from build123d import *

# Parameters (mm, degrees)
CUT_EXTRUDE1_DEPTH = 261.839989265
CHAMFER1_SIZE      = 2
FILLET1_R          = 0.5


with BuildPart() as part:
    # Sketch1 → Revolve1 (revolve)
    with BuildSketch(Plane.XY, mode=Mode.PRIVATE) as revolve1_sk:
        with BuildLine():
            Line((-125, 122.5), (-116.767790327, 122.5))
            Line((-116.767790327, 122.5), (-10.2606043, 83.734554551))
            ThreePointArc((-10.2606043, 83.734554551), (0, 81.925333174), (10.2606043, 83.734554551))
            Line((10.2606043, 83.734554551), (116.767790327, 122.5))
            Line((116.767790327, 122.5), (125, 122.5))
            Line((125, 122.5), (125, 88.250057247))
            Line((125, 88.250057247), (64.082356705, 66.077848346))
            ThreePointArc((64.082356705, 66.077848346), (59.582843437, 58.284462756), (66.476497708, 52.5))
            Line((66.476497708, 52.5), (70, 52.5))
            Line((70, 52.5), (70, 0))
            Line((70, 0), (-70, 0))
            Line((-70, 0), (-70, 52.5))
            Line((-70, 52.5), (-66.476497708, 52.5))
            ThreePointArc((-66.476497708, 52.5), (-59.582843437, 58.284462756), (-64.082356705, 66.077848346))
            Line((-64.082356705, 66.077848346), (-125, 88.250057247))
            Line((-125, 88.250057247), (-125, 122.5))
        make_face()
    revolve(revolve1_sk.sketch.rotate(Axis((-70, 0, 0), (1, 0, 0)), 90), axis=Axis((-70, 0, 0), (1, 0, 0)))

    # Sketch2 → Cut-Extrude1 (cut, through all)
    with BuildSketch(Plane.ZY.offset(70)):
        with BuildLine():
            Line((-11, 45.4), (11, 45.4))
            Line((11, 45.4), (11, 38.457769046))
            ThreePointArc((11, 38.457769046), (0, -40), (-11, 38.457769046))
            Line((-11, 38.457769046), (-11, 45.4))
        make_face()
    extrude(amount=-CUT_EXTRUDE1_DEPTH, mode=Mode.SUBTRACT)

    # Chamfer1
    chamfer1_edges = [part.edges().sort_by_distance(p)[0] for p in [
        (70, -40, 0),
        (-70, -40, 0),
    ]]
    chamfer(chamfer1_edges, length=CHAMFER1_SIZE)

    # Fillet1
    fillet1_edges = [part.edges().sort_by_distance(p)[0] for p in [
        (0, 45.4, -11),
        (0, 45.4, 11),
    ]]
    fillet(fillet1_edges, radius=FILLET1_R)


solid = part.part
Source: CAD feature listing. Evaluate the final solid. Frame: model axes, mm. A direction names the side the tool comes from. Give positions to 0.01 mm unless a question says otherwise; leave off trailing zeros. Order: outer loops, then holes, each group sorted by start corner. A loop starts at its lowest first (then second) coordinate and runs counter-clockwise, first axis right, second up. Notation, with made-up numbers: (-29.5, 77.25) -> (16.5, 77.25) arc R20 ccw to (16.5, 107.25) -> close; hole circle Ø3 at (46.5, -31). An arc over 180 degrees is marked (long way). Use a Markdown table: item, result.
1) Mould query, pull axis Y, two halves, no side actions, for faces 6 (the cylindrical face through (-0.952, -39.968, 1.603)), 7 (the flat face through (125, 80, 53)), 8 (the conical face through (-27.27, 54.72, -71.36)). Classes: +Y half, -Y half, draft (parallel to the pull), parting line (faces both ways), or undercut.
Answer list:
| item | result |
|---|---|
| face 6 | undercut |
| face 7 | draft |
| face 8 | parting line |
2) Section query B-B, the plane x = 37. Return the cut outline in (y, z), then the cut area to 3 significant figures.
Answer list:
| item | result |
|---|---|
| outline | circle Ø186.93 at (0, 0); hole (38.46, -11) -> (44.9, -11) arc R0.5 ccw to (45.4, -10.5) -> (45.4, 10.5) arc R0.5 ccw to (44.9, 11) -> (38.46, 11) arc R40 ccw (long way) to start |
| area | 22,300 mm² |
3) Contact query for flat-ended pins moving along their axis: P1, Ø7, axis at x = -19, y = 43, coming from the -Z side; P2, Ø1, axis at x = 24, z = 25, coming from the +Y side; P3, Ø12, axis at y = 53, z = -5, coming from the -X side. Output: stop coordinate, or through.
Answer list:
| item | result |
|---|---|
| P1 | z = -77.92 |
| P2 | y = 85.38 |
| P3 | x = -70 |
4) Section query C-C, the plane x = -90.5. Return the cut outline in (y, z), then the cut area to 3 significant figures.
Answer list:
| item | result |
|---|---|
| outline | circle Ø225.88 at (0, 0); hole circle Ø151.39 at (0, 0) |
| area | 22,100 mm² |
5) Reachability of faces 1 (the flat face through (70, -16, -39)), 2 (the conical face through (28.76, -27.17, 86.29)), 3 (the flat face through (-70, -16, 39)), 4 (the flat face through (-1, 42, -11)), 5 (the flat face through (-125, 53, -80)) from +Z, -Z, +X, -X, +Y, -Y: full face, straight path, thin tool, end or side. Return the list, or none.
Answer list:
| item | result |
|---|---|
| face 1 | +X |
| face 2 | none |
| face 3 | -X |
| face 4 | +X, -X |
| face 5 | +Z, -Z, -X, +Y, -Y |
6) Ray query, line 1 along Z through (x, y) = (69.5, 24); line 2 along X through (y, z) = (-43.5, -77); line 3 along Y through (x, z) = (50.5, -8). Return the intervals inside material, ascending. Write a range as [from, to].
Answer list:
| item | result |
|---|---|
| line 1 | [-102.52, -63.68], [-46.69, -33.86], [33.86, 46.69], [63.68, 102.52] |
| line 2 | [-125, -23.18], [23.18, 125] |
| line 3 | [-98.05, -39.19], [45.4, 98.05] |
